Source: CAD feature listing. Evaluate the final solid. Frame: model axes, mm. A direction names the side the tool comes from. Give positions to 0.01 mm unless a question says otherwise; leave off trailing zeros. Loops run counter-clockwise (first coordinate to the right, second up) from the corner with the lowest first, then second, coordinate; pieces in that order, holes last. Notation, with made-up numbers: M -4,36.25 L 16,36.25 A8 ccw 16,43.25 Z; hole C 34.5,36 d3. An arc over 180 degrees is marked long. Write item = value, one per line.
from build123d import *

# Parameters (mm, degrees)
CHAMFER1_SIZE = 0.5


with BuildPart() as part:
    # Sketch1 → Revolve1 (revolve)
    with BuildSketch(Plane.XY, mode=Mode.PRIVATE) as revolve1_sk:
        Polygon((131.66284067, -334.3040125), (131.66284067, -338.0040125), (129.16284067, -338.0040125), (129.16284067, -343.5040125), (126.66284067, -343.5040125), (126.66284067, -346.5040125), (136.66284067, -346.5040125), (136.66284067, -334.3040125), align=None)
    revolve(revolve1_sk.sketch.rotate(Axis((136.66284067, -346.5040125, 0), (0, 1, 0)), 270), axis=Axis((136.66284067, -346.5040125, 0), (0, 1, 0)))

    # Chamfer1
    chamfer1_edges = [part.edges().sort_by_distance(p)[0] for p in [
        (136.66284067, -334.3040125, 5),
        (136.66284067, -346.5040125, 10),
        (136.66284067, -343.5040125, 10),
        (136.66284067, -338.0040125, 7.5),
    ]]
    chamfer(chamfer1_edges, length=CHAMFER1_SIZE)


solid = part.part
1. Reachability of faces 1 (the flat face through (129, -343.504, 1)), 2 (the cylindrical face through (146.425, -345.018, 2.168)) from +Z, -Z, +X, -X, +Y, -Y: full face, straight path, thin tool, end or side. Return the list, or none.
Derived:
face_1 = +Y
face_2 = +Y, -Y
2. First-contact query: pin 1 Ø1.5 at (x, y) = (133.5, -337) entering from -Z; pin 2 Ø4 at (y, z) = (-340, -1.5) entering from -X; pin 3 Ø3 at (x, y) = (134, -342.5) entering from +Z. Flat tips, straight axial feed; report the tip coordinate or a pass-through.
Derived:
pin_1 = -4.38
pin_2 = 129.16
pin_3 = 9.68
3. Cut plane C-C, the plane y = -345. Return the cut outline in (x, z), then the cut area to 3 significant figures.
Derived:
outline = C 136.66,0 d20
area = 314 mm²
4. Cut plane B-B, the plane y = -336.5. Return the cut outline in (x, z), then the cut area to 3 significant figures.
Derived:
outline = C 136.66,0 d10
area = 78.5 mm²
5. Cut plane A-A, the plane z = 0. Return the cut outline in (x, y).
Derived:
outline = M 126.66,-346 L 127.16,-346.5 L 146.16,-346.5 L 146.66,-346 L 146.66,-344 L 146.16,-343.5 L 144.16,-343.5 L 144.16,-338.5 L 143.66,-338 L 141.66,-338 L 141.66,-334.8 L 141.16,-334.3 L 132.16,-334.3 L 131.66,-334.8 L 131.66,-338 L 129.66,-338 L 129.16,-338.5 L 129.16,-343.5 L 127.16,-343.5 L 126.66,-344 Z
6. Material intervals for probe 1 along Y at (x, z) = (143.25, -3.75); probe 2 along Y at (x, z) = (140.25, 5); probe 3 along Z at (x, y) = (136.75, -338.75), sorted ascending. Write a range as from..to.
Derived:
probe_1 = -346.5..-343.5
probe_2 = -346.5..-338
probe_3 = -7.5..7.5
